```python
from build123d import *

# Parameters (mm, degrees)
SKETCH_1_W             = 248
SKETCH_1_H             = 60
EXTRUDE_1_DEPTH        = 6
EXTRUDE_2_DEPTH        = 12
FILLET_1_R             = 20
SKETCH_3_R             = 40
CUT_EXTRUDE_1_DEPTH    = 319.384987083
HOLE_WIZARD_M5_1_D     = 4.2
HOLE_WIZARD_M5_1_DEPTH = 12.4
HOLE_WIZARD_M5_1_TIP   = 1.2618073
HOLE_WIZARD_M5_2_D     = 4.2
HOLE_WIZARD_M5_2_DEPTH = 12.4
HOLE_WIZARD_M5_2_TIP   = 1.2618073


with BuildPart() as part:
    # 草图1 → 凸台-拉伸1 (new, symmetric)
    with BuildSketch(Plane.XY):
        Rectangle(SKETCH_1_W, SKETCH_1_H)
    extrude(amount=EXTRUDE_1_DEPTH, both=True)

    # 草图2 → 凸台-拉伸2 (add)
    with BuildSketch(Plane(origin=(0, 0, -6), x_dir=(-1, 0, 0), z_dir=(0, 0, -1))):
        Polygon((-124, 30), (74, 180), (74, 293), (124, 293), (124, 30), align=None)
    extrude(amount=-EXTRUDE_2_DEPTH)

    # 圆角1
    fillet_1_edges = [part.edges().sort_by_distance(p)[0] for p in [
        (-74, 180, 0),
    ]]
    fillet(fillet_1_edges, radius=FILLET_1_R)

    # 草图3 → 切除-拉伸1 (cut, through all)
    with BuildSketch(Plane(origin=(0, 0, -6), x_dir=(-1, 0, 0), z_dir=(0, 0, -1))):
        with Locations((-26, 20)):
            Circle(SKETCH_3_R)
        with Locations((64, 90)):
            Circle(SKETCH_3_R)
    extrude(amount=-CUT_EXTRUDE_1_DEPTH, mode=Mode.SUBTRACT)

    # M5 螺纹孔1
    with Locations(Plane(origin=(0, -30, 0), x_dir=(-1, 0, 0), z_dir=(0, -1, 0))):
        with Locations((-90, 0), (0, 0), (90, 0)):
            Hole(HOLE_WIZARD_M5_1_D / 2, depth=HOLE_WIZARD_M5_1_DEPTH)
            with Locations((0, 0, -(HOLE_WIZARD_M5_1_DEPTH + HOLE_WIZARD_M5_1_TIP / 2))):  # 118° drill point
                Cone(0, HOLE_WIZARD_M5_1_D / 2, HOLE_WIZARD_M5_1_TIP, mode=Mode.SUBTRACT)

    # M5 螺纹孔2
    with Locations(Plane.ZY.offset(124)):
        with Locations((0, 238), (0, 128), (0, 18)):
            Hole(HOLE_WIZARD_M5_2_D / 2, depth=HOLE_WIZARD_M5_2_DEPTH)
            with Locations((0, 0, -(HOLE_WIZARD_M5_2_DEPTH + HOLE_WIZARD_M5_2_TIP / 2))):  # 118° drill point
                Cone(0, HOLE_WIZARD_M5_2_D / 2, HOLE_WIZARD_M5_2_TIP, mode=Mode.SUBTRACT)


solid = part.part
```
Read the model definition and answer for the solid it produces. Units are mm, in the model's axes. A direction names the side the tool comes from. Coordinates: 2 decimals unless noted, no trailing zeros. Write each loop counter-clockwise with the first axis right and the second up, starting at its lowest first coordinate (ties: lowest second). Pieces come first, ordered by that corner, then holes. Notation, with made-up numbers: (-3.5, -4.5) -> (41.5, -4.5) arc R18 ccw to (41.5, 0.5) -> close; hole circle Ø10 at (20.5, 81.5). An arc over 180 degrees is marked (long way). Answer as a JSON object with one key per item and string values.
Q1. Flat-ended cylindrical pins translate along their axes: pin 1 Ø4 at (x, z) = (0, 0) entering from +Y; pin 2 Ø6 at (y, z) = (265.5, 2) entering from +X; pin 3 Ø6.5 at (x, z) = (90, 0) entering from +Y. Find the tip coordinate at first contact, or state that the pin passes through.
The answers:
{"pin 1": "stops at y = 125.45", "pin 2": "stops at x = -74", "pin 3": "stops at y = 58.22"}
Q2. A tool of negligible diameter and unlimited length cuts with its end or side. For faces 1 (the flat face through (-74, 241, 0)), 2 (the cylindrical face through (-102.153, 102.015, -0.084)), from which of +Z, -Z, +X, -X, +Y, -Y can it reach the whole face along a straight path? Write none if from no direction.
The answers:
{"face 1": "+Z, -Z, +X, +Y", "face 2": "+Z, -Z"}
Q3. Consider line 1 (Y direction, x = -117, z = 0); line 2 (Z direction, x = -120, y = 238); line 3 (X direction, y = 219.5, z = -5.25). Determine where each line is inside the solid, lowest interval first. Write a range as [from, to].
The answers:
{"line 1": "y = [-30, 15.9], [20.1, 125.9], [130.1, 235.9], [240.1, 293]", "line 2": "z = [-6, -2.1], [2.1, 6]", "line 3": "x = [-124, -74]"}
Q4. Determine the mould class of faces 3 (the flat face through (-29, 62, 6)), 4 (the cylindrical face through (31.21, 59.66, -0.08)), 5 (the cylindrical face through (-71.85, 180.92, 0.08)) for opening direction X: pulls with the +X half, pulls with the -X half, needs draft (parallel to the pull), parting line crosses it, or undercut.
The answers:
{"face 3": "needs draft", "face 4": "undercut", "face 5": "pulls with the +X half"}
Q5. The part is cut by section C-C on x = 38. Give the vertices of the cut face in (y, z), then the cut area to 3 significant figures.
The answers:
{"outline": "(-30, -6) -> (-18.16, -6) -> (-18.16, 6) -> (-30, 6) -> close; (58.16, -6) -> (95.15, -6) -> (95.15, 6) -> (58.16, 6) -> close", "area": "586 mm2"}
Q6. The part is cut by section D-D on y = 206. Give the vertices of the cut face in (x, z), then the cut area to 3 significant figures.
The answers:
{"outline": "(-124, -6) -> (-74, -6) -> (-74, 6) -> (-124, 6) -> close", "area": "600 mm2"}
Q7. The part is cut by section A-A on z = -4. Give the vertices of the cut face in (x, y), then the cut area to 3 significant figures.
The answers:
{"outline": "(-124, -30) -> (124, -30) -> (124, 30) -> (-66.08, 174) arc R20 cw to (-74, 189.94) -> (-74, 293) -> (-124, 293) -> close; hole circle Ø80 at (-64, 90); hole circle Ø80 at (26, 20)", "area": "32,800 mm2"}
Q8. The part is cut by section B-B on y = 122. Give the vertices of the cut face in (x, z), then the cut area to 3 significant figures.
The answers:
{"outline": "(-124, -6) -> (-88, -6) -> (-88, 6) -> (-124, 6) -> close; (-40, -6) -> (2.56, -6) -> (2.56, 6) -> (-40, 6) -> close", "area": "943 mm2"}
